```python
from build123d import *


with BuildPart() as part:
    # Sketch1 → Revolve1 (revolve)
    with BuildSketch(Plane.XY, mode=Mode.PRIVATE) as revolve1_sk:
        Polygon((3.5, 20), (0, 16.5), (-3.5, 20), (-7.5, 20), (-7.5, 16.5), (-2.5, 16.5), (-2.5, 5), (-7.5, 5), (-7.5, 3.125), (7.5, 3.125), (7.5, 5), (2.5, 5), (2.5, 16.5), (7.5, 16.5), (7.5, 20), align=None)
    revolve(revolve1_sk.sketch.rotate(Axis((-45.5, 0, 0), (1, 0, 0)), 90), axis=Axis((-45.5, 0, 0), (1, 0, 0)))


solid = part.part
```
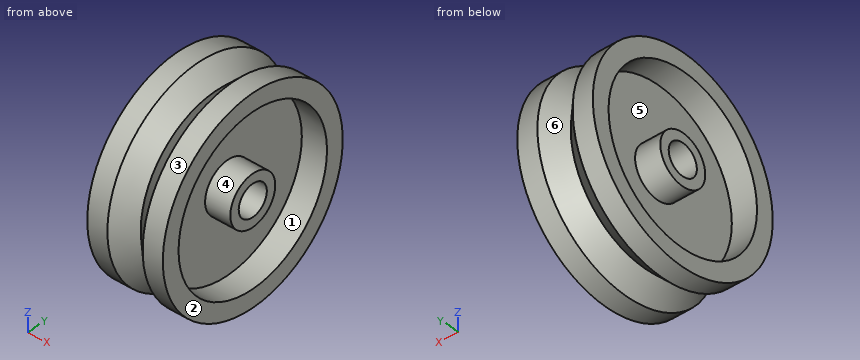
Work out the finished part from the listing and answer in its coordinate system (mm). Face numbers are marked on the shaded views. A direction names the side the tool comes from. Round coordinates to 2 decimals unless told otherwise and drop trailing zeros. Write each loop counter-clockwise with the first axis right and the second up, starting at its lowest first coordinate (ties: lowest second). Pieces come first, ordered by that corner, then holes.
1) Flat-ended cylindrical pins translate along their axes: P1, Ø2, axis at y = -3, z = 8, coming from the -X side; P2, Ø2, axis at x = -4.5, z = 15.5, coming from the -Y side (3 decimals); P3, Ø3, axis at x = -6, z = 8, coming from the -Y side; P4, Ø10, axis at y = -0.5, z = 0, coming from the -X side. Find the tip coordinate at first contact, or state that the pin passes through.
2) Which of the six approach directions +Z, -Z, +X, -X, +Y, -Y give full straight-line access (tool end or side, diameter ignored) to the marked faces 4, 5 and 6?
3) Determine the mould class of the marked faces 1, 2 and 3 for opening direction Y: pulls with the +Y half, pulls with the -Y half, needs draft (parallel to the pull), parting line crosses it, or undercut.
4) Consider probe 1 along Y at (x, z) = (-5.15, 0) (3 decimals); probe 2 along X at (y, z) = (-7.5, 11.5); probe 3 along Y at (x, z) = (-3.5, 14). Determine where each line is inside the solid, lowest interval first.
5) A cutting plane is placed at D-D on x = -1.75. Determine the outline of the cut face in (y, z) (3 decimals).
6) A cutting plane is placed at B-B on x = -6. Determine the outline of the cut face in (y, z) (3 decimals).
Entries:
1. P1: stops at x = -2.5
1. P2: stops at y = -13.775
1. P3: stops at y = -18.91
1. P4: stops at x = -7.5
2. face 4: +X
2. face 5: -X
2. face 6: none
3. face 1: undercut
3. face 2: needs draft
3. face 3: parting line crosses it
4. probe 1: y = -20 to -16.5, -5 to -3.125, 3.125 to 5, 16.5 to 20
4. probe 2: x = -2.5 to 2.5
4. probe 3: y = -14.28 to -8.73, 8.73 to 14.28
5. outline: circle Ø36.5 at (0, 0); hole circle Ø6.25 at (0, 0)
6. outline: circle Ø40 at (0, 0); circle Ø10 at (0, 0); hole circle Ø33 at (0, 0); hole circle Ø6.25 at (0, 0)
